Input: part model. Units: mm. Frame: model coordinates. A direction names the side the tool comes from. Coordinates: 2 decimals unless noted, no trailing zeros. Loops run counter-clockwise (first coordinate to the right, second up) from the corner with the lowest first, then second, coordinate; pieces in that order, holes last.
(1) Section B-B, the plane y = 88. Return loops of the section in (x, z), then the cut area to 3 significant figures.
(2) Section C-C, the plane z = 28. Return loops of the section in (x, y), then the cut area to 3 significant figures.
(3) Mould query, pull axis X, two halves, no side actions, for faces 6 (the face through (75, 57, 15)), 7 (the face through (15.1, 112.5, 12.5)), 8 (the face through (28, 54, 0)). Classes: released by +X, released by -X, zero draft, split by the parting line, or undercut.
(4) Section A-A, the plane x = 37.5. Return loops of the section in (y, z).
(5) Line query: L1, parallel to Z at x = 10, y = 2.7; L2, parallel to Y at x = 38, z = 4.25; L3, parallel to X at y = 77.5, z = 27.25. Output: solid intervals per line, ascending.
(6) Contact query for flat-ended pins moving along their axis: P1, Ø16.5, axis at x = 86, z = 9.5, coming from the -Y side; P2, Ø1.5, axis at y = 112, z = 19.5, coming from the -X side; P3, Ø9, axis at y = 78.5, z = 17.5, coming from the -X side; P4, Ø4, axis at y = 113.5, z = 15, coming from the +X side. Output: stop coordinate, or through.
(7) Set-up query: faces 1 (the face through (85, 5, 15)), 2 (the face through (87.48, 112.54, 14.67)), 3 (the face through (10, 113, 15)), 4 (the face through (92.95, 2.54, 17.7)), 5 (the face through (30, 57, 15)). Return all of +Z, -Z, +X, -X, +Y, -Y with unobstructed straight access to the full face (end or side cutting, diameter ignored); none if empty.
```python
from build123d import *

# Parameters (mm, degrees)
SKETCH1_W           = 40
SKETCH1_H           = 105
BOSS_EXTRUDE1_DEPTH = 30
SKETCH2_R           = 4
CUT_EXTRUDE1_DEPTH  = 152.657508881
SKETCH3_R           = 2.5
CUT_EXTRUDE2_DEPTH  = 10


with BuildPart() as part:
    # Sketch1 → Boss-Extrude1 (new body)
    with BuildSketch(Plane.XY):
        Polygon((0, 0), (100, 0), (100, 5), (75, 5), (75, 110), (90, 110), (90, 115), (10, 115), (10, 110), (25, 110), (25, 5), (0, 5), align=None)
        with Locations((50, 57.5)):
            Rectangle(SKETCH1_W, SKETCH1_H, mode=Mode.SUBTRACT)
    extrude(amount=BOSS_EXTRUDE1_DEPTH)

    # Sketch2 → Cut-Extrude1 (cut, through all)
    with BuildSketch(Plane(origin=(0, 5, 0), x_dir=(1, 0, 0), z_dir=(0, 1, 0))):
        with Locations(Location((90, -15, 0), (0, 0, 180))):
            Circle(SKETCH2_R)
        with Locations(Location((10, -15, 0), (0, 0, 180))):
            Circle(SKETCH2_R)
    extrude(amount=-CUT_EXTRUDE1_DEPTH, mode=Mode.SUBTRACT)

    # Sketch3 → Cut-Extrude2 (cut)
    with BuildSketch(Plane(origin=(0, 115, 0), x_dir=(1, 0, 0), z_dir=(0, 1, 0))):
        with Locations(Location((15, -15, 0), (0, 0, 270))):
            Circle(SKETCH3_R)
        with Locations(Location((85, -15, 0), (0, 0, 270))):
            Circle(SKETCH3_R)
    extrude(amount=-CUT_EXTRUDE2_DEPTH, mode=Mode.SUBTRACT)


solid = part.part
```
Report:
1. outline: (25, 0) - (30, 0) - (30, 30) - (25, 30) - close; (70, 0) - (75, 0) - (75, 30) - (70, 30) - close
1. area: 300 mm2
2. outline: (0, 0) - (100, 0) - (100, 5) - (75, 5) - (75, 110) - (90, 110) - (90, 115) - (10, 115) - (10, 110) - (25, 110) - (25, 5) - (0, 5) - close; hole (30, 5) - (70, 5) - (70, 110) - (30, 110) - close
2. area: 1,950 mm2
3. face 6: released by +X
3. face 7: undercut
3. face 8: zero draft
4. outline: (0, 0) - (5, 0) - (5, 30) - (0, 30) - close; (110, 0) - (115, 0) - (115, 30) - (110, 30) - close
5. L1: z = 0 to 11, 19 to 30
5. L2: y = 0 to 5, 110 to 115
5. L3: x = 25 to 30, 70 to 75
6. P1: stops at y = 0
6. P2: stops at x = 10
6. P3: stops at x = 25
6. P4: stops at x = 90
7. face 1: +Z, -Z, +X
7. face 2: +Y
7. face 3: +Z, -Z, -X, +Y
7. face 4: -Y
7. face 5: +Z, -Z
